Could you check a few things on this model? Use its own coordinates, in mm. A direction names the side the tool comes from. Give positions to 0.01 mm unless a question says otherwise; leave off trailing zeros. Loops run counter-clockwise (first coordinate to the right, second up) from the corner with the lowest first, then second, coordinate; pieces in that order, holes last. Notation, with made-up numbers: M 61.5,79.5 L 67.5,79.5 A17 cw 67.5,85.5 Z; hole C 7,-26.75 d5. An arc over 180 degrees is marked long. Use CSV: the item, a comma, the result in double quotes.
```python
from build123d import *

# Parameters (mm, degrees)
SKETCH1_W           = 30
SKETCH1_H           = 35
SKETCH1_R           = 3.5
SKETCH1_R_2         = 1.5
BOSS_EXTRUDE1_DEPTH = 3
SKETCH2_W           = 30
SKETCH2_H           = 4
BOSS_EXTRUDE2_DEPTH = 15
SKETCH4_R           = 1.5
CUT_EXTRUDE1_DEPTH  = 15


with BuildPart() as part:
    # Sketch1 → Boss-Extrude1 (new body)
    with BuildSketch(Plane.XY):
        Rectangle(SKETCH1_W, SKETCH1_H)
        Circle(SKETCH1_R, mode=Mode.SUBTRACT)
        with Locations((0, 7)):
            Circle(SKETCH1_R_2, mode=Mode.SUBTRACT)
        with Locations(Location((0, -7, 0), (0, 0, 180))):
            Circle(SKETCH1_R_2, mode=Mode.SUBTRACT)
    extrude(amount=BOSS_EXTRUDE1_DEPTH)

    # Sketch2 → Boss-Extrude2 (add)
    with BuildSketch(Plane.XY.offset(3)):
        with Locations((0, 15.5)):
            Rectangle(SKETCH2_W, SKETCH2_H)
        with Locations((0, -15.5)):
            Rectangle(SKETCH2_W, SKETCH2_H)
    extrude(amount=BOSS_EXTRUDE2_DEPTH)

    # Sketch4 → Cut-Extrude1 (cut)
    with BuildSketch(Plane.XZ.offset(-13.5)):
        with Locations(Location((-10, 15, 0), (0, 0, 270))):
            Circle(SKETCH4_R)
        with Locations(Location((10, 15, 0), (0, 0, 270))):
            Circle(SKETCH4_R)
        with Locations(Location((10, 7.5, 0), (0, 0, 270))):
            Circle(SKETCH4_R)
        with Locations(Location((-10, 7.5, 0), (0, 0, 270))):
            Circle(SKETCH4_R)
    cut_extrude1 = extrude(amount=-CUT_EXTRUDE1_DEPTH, mode=Mode.SUBTRACT)

    # Mirror1: Cut-Extrude1 across plane
    add(cut_extrude1.mirror(Plane.ZX), mode=Mode.SUBTRACT)


solid = part.part
```
1. Please list where these lines run through material, in increasing order: line 1 (Z direction, x = -10, y = -14.5); line 2 (Y direction, x = 0, z = 0.9); line 3 (X direction, y = -15.35, z = 15).
Outcome:
line 1,"0 to 6, 9 to 13.5, 16.5 to 18"
line 2,"-17.5 to -8.5, -5.5 to -3.5, 3.5 to 5.5, 8.5 to 17.5"
line 3,"-15 to -11.5, -8.5 to 8.5, 11.5 to 15"
2. I want a section at D-D, the plane x = 10. List the corners of the cut face in (y, z) for me.
Outcome:
outline,"M -17.5,0 L 17.5,0 L 17.5,6 L 13.5,6 L 13.5,3 L -13.5,3 L -13.5,6 L -17.5,6 Z; M -17.5,9 L -13.5,9 L -13.5,13.5 L -17.5,13.5 Z; M -17.5,16.5 L -13.5,16.5 L -13.5,18 L -17.5,18 Z; M 13.5,9 L 17.5,9 L 17.5,13.5 L 13.5,13.5 Z; M 13.5,16.5 L 17.5,16.5 L 17.5,18 L 13.5,18 Z"
3. I want a section at A-A, the plane z = 3.75. List the corners of the cut face in (x, y) for me, then the cut area to 3 significant figures.
Outcome:
outline,"M -15,-17.5 L 15,-17.5 L 15,-13.5 L -15,-13.5 Z; M -15,13.5 L 15,13.5 L 15,17.5 L -15,17.5 Z"
area,"240 mm2"
4. I'm going to push a flat-ended pin straight in: pin 1 Ø1.5 at (x, y) = (1, 5.5) entering from +Z. Where does the tip first touch, or does it pass through?
Outcome:
pin 1,"z = 3"
5. Which directions (+Z, -Z, +X, -X, +Y, -Y) give clear straight access to the entire face, cutting with the end or side of a thin tool? Please do faces 5 (the face through (15, 0, 1)), 6 (the face through (-4, 0, 3)).
Outcome:
face 5,"+Z, -Z, +X, +Y, -Y"
face 6,"+Z, +X, -X"
6. I want a section at B-B, the plane x = 0. List the corners of the cut face in (y, z) for me.
Outcome:
outline,"M -17.5,0 L -8.5,0 L -8.5,3 L -13.5,3 L -13.5,18 L -17.5,18 Z; M -5.5,0 L -3.5,0 L -3.5,3 L -5.5,3 Z; M 3.5,0 L 5.5,0 L 5.5,3 L 3.5,3 Z; M 8.5,0 L 17.5,0 L 17.5,18 L 13.5,18 L 13.5,3 L 8.5,3 Z"
7. I want a section at C-C, the plane y = 7. List the corners of the cut face in (x, z) for me, then the cut area to 3 significant figures.
Outcome:
outline,"M -15,0 L -1.5,0 L -1.5,3 L -15,3 Z; M 1.5,0 L 15,0 L 15,3 L 1.5,3 Z"
area,"81.0 mm2"
8. If we mould it in two halves opening along Y, with no side actions, what happens to faces 1 (the face through (-0.325, 5.536, 1.479)), 2 (the face through (0, -17.5, 9)), 3 (the face through (0, 17.5, 9)), 4 (the face through (-10.9, -15.5, 8.7))? For each: +Y half, -Y half, draft (parallel to the pull), parting line (faces both ways), or undercut.
Outcome:
face 1,"undercut"
face 2,"-Y half"
face 3,"+Y half"
face 4,"draft"
